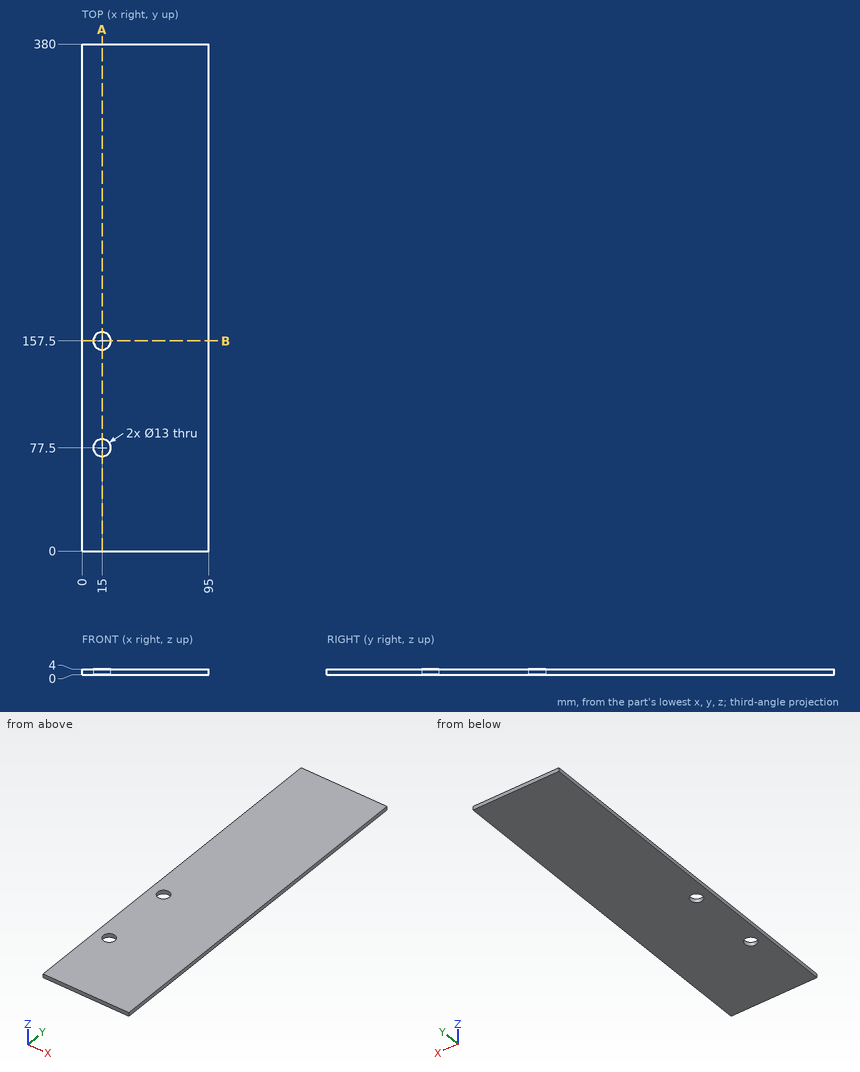
Answer from the drawing. Dimensions are ordinates in mm from the lowest x, y and z of the part. Round coordinates to 2 decimals unless told otherwise and drop trailing zeros. Loops run counter-clockwise (first coordinate to the right, second up) from the corner with the lowest first, then second, coordinate; pieces in that order, holes last.
(1) The part is cut by section B-B, the plane y = 157.5. Give the vertices of the cut face in (x, z).
Computed values:
outline: (0, 0) - (8.5, 0) - (8.5, 4) - (0, 4) - close; (21.5, 0) - (95, 0) - (95, 4) - (21.5, 4) - close
(2) The part is cut by section A-A, the plane x = 15. Give the vertices of the cut face in (y, z), and give its area (3 significant figures).
Computed values:
outline: (0, 0) - (71, 0) - (71, 4) - (0, 4) - close; (84, 0) - (151, 0) - (151, 4) - (84, 4) - close; (164, 0) - (380, 0) - (380, 4) - (164, 4) - close
area: 1,420 mm2
(3) This flat-tipped pin is pushed along its axis until it touches: P1, Ø11.5, axis at x = 15, y = 157.5, coming from the -Z side. Where does it stop, or does it pass through?
Computed values:
P1: passes through
(4) Find the intervals of material crossed by L1, parallel to Y at x = 15, z = 1.7, in increasing order.
Computed values:
L1: y = 0 to 71, 84 to 151, 164 to 380
